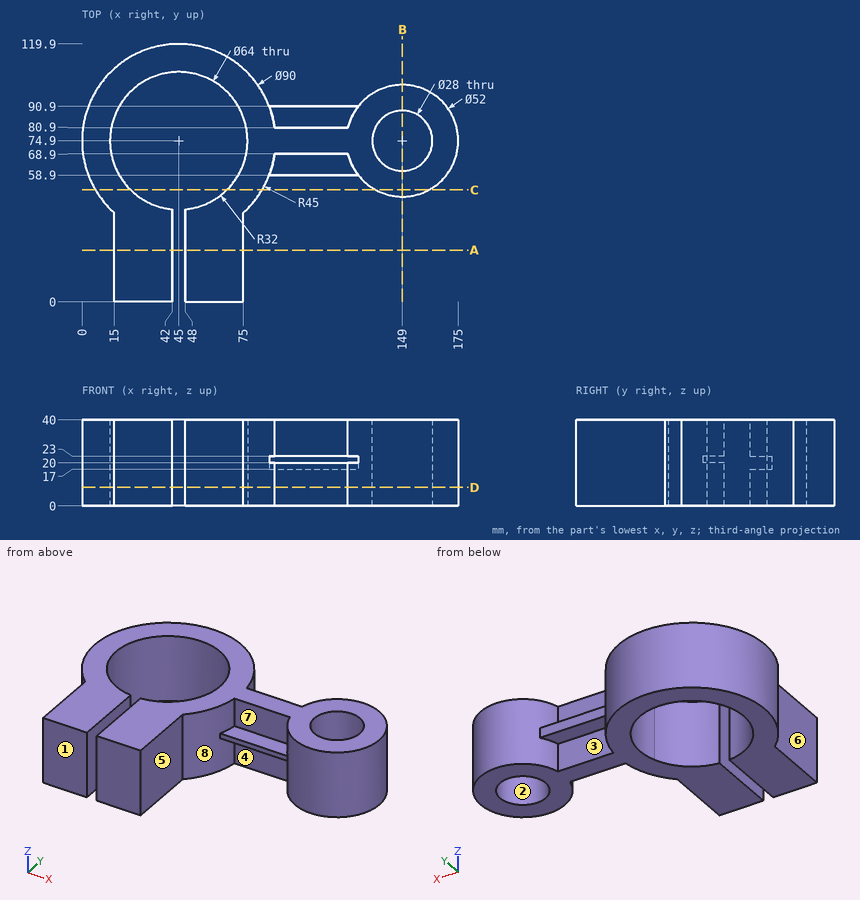
Input: dimensioned drawing with shaded views. Units: mm. Origin: part minimum x, y, z. A direction names the side the tool comes from. Round coordinates to 2 decimals unless told otherwise and drop trailing zeros. Write each loop counter-clockwise with the first axis right and the second up, starting at its lowest first coordinate (ties: lowest second). Pieces come first, ordered by that corner, then holes. Notation, with made-up numbers: (87.25, -10.5) - (121.25, -10.5) arc R24 ccw to (121.25, 14.5) - close; hole circle Ø1 at (20, -25). An arc over 180 degrees is marked (long way). Write item = value, one per line.
(1) Pull-direction query (Y, two-part tool) for the marked faces 1, 2 and 3; classes: +Y half, -Y half, draft (parallel to the pull), parting line (faces both ways), or undercut.
Geometry check:
face_1 = -Y half
face_2 = undercut
face_3 = +Y half
(2) Section query D-D on z = 8.5. Output: boundary loops of the cut face in (x, y).
Geometry check:
outline = (15, 0) - (42, 0) - (42, 43.04) arc R32 cw (long way) to (48, 43.04) - (48, 0) - (75, 0) - (75, 41.36) arc R45 ccw to (89.6, 68.9) - (123.7, 68.9) arc R26 ccw (long way) to (123.7, 80.9) - (89.6, 80.9) arc R45 ccw (long way) to (15, 41.36) - close; hole circle Ø28 at (149, 74.9)
(3) Access query for the marked faces 4, 5, 6, 7 and 8. Directions: +Z, -Z, +X, -X, +Y, -Y. A direction counts if a zero-diameter tool reaches every point of the face in a straight line with its end or side. Return the directions, or none.
Geometry check:
face_4 = -Z, -Y
face_5 = +Z, -Z, +X, -Y
face_6 = +Z, -Z, -X, -Y
face_7 = +Z, -Y
face_8 = -Y
(4) Contact query for flat-ended pins moving along their axis: pin 1 Ø18.5 at (x, z) = (105.5, 7.5) entering from +Y; pin 2 Ø4 at (x, z) = (52.5, 28.5) entering from +Y; pin 3 Ø6.5 at (x, z) = (110, 20.5) entering from +Y. Output: stop coordinate, or through.
Geometry check:
pin_1 = 80.9
pin_2 = 119.56
pin_3 = 90.9
(5) Section query C-C on y = 52. Output: boundary loops of the cut face in (x, z).
Geometry check:
outline = (6.26, 0) - (22.65, 0) - (22.65, 40) - (6.26, 40) - close; (67.35, 0) - (83.74, 0) - (83.74, 40) - (67.35, 40) - close; (136.69, 0) - (161.31, 0) - (161.31, 40) - (136.69, 40) - close
(6) Material intervals for probe 1 along X at (y, z) = (35, 37.5); probe 2 along X at (y, z) = (98, 36.5) (1 decimal); probe 3 along X at (y, z) = (60, 9.5), sorted ascending.
Geometry check:
probe_1 = 15 to 42, 48 to 75
probe_2 = 6.4 to 22.9, 67.1 to 83.6, 137.1 to 160.9
probe_3 = 2.54 to 16.68, 73.32 to 87.46, 127.69 to 170.31
(7) Section query A-A on y = 24. Output: boundary loops of the cut face in (x, z), then the cut area to 3 significant figures.
Geometry check:
outline = (15, 0) - (42, 0) - (42, 40) - (15, 40) - close; (48, 0) - (75, 0) - (75, 40) - (48, 40) - close
area = 2,160 mm^2
(8) Section query B-B on x = 149. Output: boundary loops of the cut face in (y, z), then the cut area to 3 significant figures.
Geometry check:
outline = (48.9, 0) - (60.9, 0) - (60.9, 40) - (48.9, 40) - close; (88.9, 0) - (100.9, 0) - (100.9, 40) - (88.9, 40) - close
area = 960 mm^2
